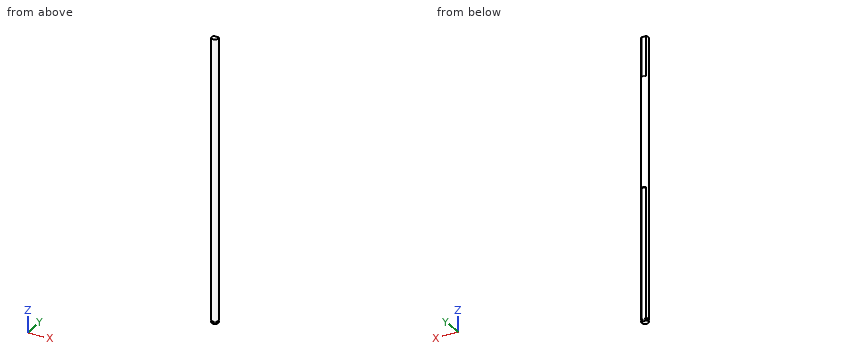
from build123d import *

# Parameters (mm, degrees)
SKETCH1_R           = 2.5
BOSS_EXTRUDE1_DEPTH = 213
CUT_EXTRUDE2_DEPTH  = 100
CUT_EXTRUDE3_START  = 1
SKETCH5_R           = 2.5
SKETCH5_R_2         = 2
CUT_EXTRUDE3_DEPTH  = 1
CUT_EXTRUDE4_START  = -30
CUT_EXTRUDE4_DEPTH  = 30


with BuildPart() as part:
    # Sketch1 → Boss-Extrude1 (new body)
    with BuildSketch(Plane.XY):
        Circle(SKETCH1_R)
    extrude(amount=BOSS_EXTRUDE1_DEPTH)

    # Sketch4 → Cut-Extrude2 (cut)
    with BuildSketch(Plane(origin=(0, 0, 0), x_dir=(-1, 0, 0), z_dir=(0, 0, -1))):
        with BuildLine():
            Line((-1.833030278, 1.7), (1.833030278, 1.7))
            ThreePointArc((1.833030278, 1.7), (0, 2.5), (-1.833030278, 1.7))
        make_face()
    extrude(amount=-CUT_EXTRUDE2_DEPTH, mode=Mode.SUBTRACT)

    # Sketch5 → Cut-Extrude3 (cut)
    with BuildSketch(Plane(origin=(0, 0, 2), x_dir=(-1, 0, 0), z_dir=(0, 0, -1)).offset(CUT_EXTRUDE3_START)):
        with Locations(Location((0, 0, 0), (0, 0, 42.843643044))):
            Circle(SKETCH5_R)
        Circle(SKETCH5_R_2, mode=Mode.SUBTRACT)
    extrude(amount=-CUT_EXTRUDE3_DEPTH, mode=Mode.SUBTRACT)

    # Sketch7 → Cut-Extrude4 (cut)
    with BuildSketch(Plane.XY.offset(213).offset(CUT_EXTRUDE4_START)):
        with BuildLine():
            Line((-1.835, 1.69787367), (1.835, 1.69787367))
            ThreePointArc((1.835, 1.69787367), (0, 2.5), (-1.835, 1.69787367))
        make_face()
    extrude(amount=CUT_EXTRUDE4_DEPTH, mode=Mode.SUBTRACT)


solid = part.part
Geometry check sheet. Reference: the model listing, model coordinates, mm. Round coordinates to 2 decimals unless told otherwise and drop trailing zeros. Loops run counter-clockwise (first coordinate to the right, second up) from the corner with the lowest first, then second, coordinate; pieces in that order, holes last.
Item 1: Cross-section at C-C on z = 55. Record the boundary of the cut face in (x, y), then the cut area to 3 significant figures.
Item 2: Cross-section at B-B on z = 197. Record the boundary of the cut face in (x, y) (3 decimals), then the cut area to 3 significant figures.
Item 3: Cross-section at A-A on x = 0. Record the boundary of the cut face in (y, z), then the cut area to 3 significant figures.
Item 4: Gauge pin test, flat ends, axial feed: pin 1 (1 mm diameter, centred on x = -0.5, y = -1, fed in from -Z); pin 2 (1.8 mm diameter, centred on x = 0.5, z = 60, fed in from +Y); pin 3 (1 mm diameter, centred on y = -1.5, z = 102.5, fed in from -X). Record the tip position at first contact, or that the pin passes through.
Item 5: Thickness scan on line 1 (Z direction, x = 0.9, y = 1.85); line 2 (Y direction, x = 1.7, z = 12.5); line 3 (Y direction, x = -0.45, z = 35.5). Record the ranges inside material, lowest first.
Item 6: Cross-section at D-D on z = 141. Record the boundary of the cut face in (x, y), then the cut area to 3 significant figures.
Answer sheet:
1. outline: (-1.83, 1.7) arc R2.5 ccw (long way) to (1.83, 1.7) - close
1. area: 17.6 mm2
2. outline: (-1.835, 1.698) arc R2.5 ccw (long way) to (1.835, 1.698) - close
2. area: 17.6 mm2
3. outline: (-2.5, 0) - (1.7, 0) - (1.7, 100) - (2.5, 100) - (2.5, 183) - (1.7, 183) - (1.7, 213) - (-2.5, 213) - (-2.5, 2) - (-2, 2) - (-2, 1) - (-2.5, 1) - close
3. area: 960 mm2
4. pin 1: stops at z = 0
4. pin 2: stops at y = 1.7
4. pin 3: stops at x = -2.29
5. line 1: z = 100 to 183
5. line 2: y = -1.83 to 1.7
5. line 3: y = -2.46 to 1.7
6. outline: circle Ø5 at (0, 0)
6. area: 19.6 mm2
